from build123d import *

# Parameters (mm, degrees)
BOSS_EXTRUDE1_DEPTH = 8
CHAMFER1_SIZE       = 15


with BuildPart() as part:
    # Sketch1 → Boss-Extrude1 (new, symmetric)
    with BuildSketch(Plane.XY):
        Polygon((0, 0), (0, 30), (340, 30), (340, 10), align=None)
    extrude(amount=BOSS_EXTRUDE1_DEPTH, both=True)

    # Chamfer1
    chamfer1_edges = [part.edges().sort_by_distance(p)[0] for p in [
        (0, 30, 0),
    ]]
    chamfer(chamfer1_edges, length=CHAMFER1_SIZE)


solid = part.part
Geometry check sheet. Reference: the model listing, model coordinates, mm. Give positions to 0.01 mm unless a question says otherwise; leave off trailing zeros. Write each loop counter-clockwise with the first axis right and the second up, starting at its lowest first coordinate (ties: lowest second). Pieces come first, ordered by that corner, then holes.
1) Thickness scan on line 1 (Y direction, x = 274, z = -3.75); line 2 (Y direction, x = 272.5, z = 0.5); line 3 (X direction, y = 18.25, z = 5.5). Record the ranges inside material, lowest first.
Values follow:
line 1: y = 8.06 to 30
line 2: y = 8.01 to 30
line 3: x = 3.25 to 340
2) Cross-section at C-C (z = 1.25). Record the boundary of the cut face in (x, y).
Values follow:
outline: (0, 0) - (340, 10) - (340, 30) - (15, 30) - (0, 15) - close
3) Cross-section at A-A (x = 42.5). Record the boundary of the cut face in (y, z).
Values follow:
outline: (1.25, -8) - (30, -8) - (30, 8) - (1.25, 8) - close
4) Go/stop test with flat-tipped pins: pin 1 Ø1 at (y, z) = (19, -0.5) entering from -X; pin 2 Ø8 at (x, z) = (241, 1.5) entering from -Y. Record where each tip stops, or that it passes through.
Values follow:
pin 1: stops at x = 3.5
pin 2: stops at y = 6.97
5) Cross-section at B-B (y = 23). Record the boundary of the cut face in (x, z).
Values follow:
outline: (8, -8) - (340, -8) - (340, 8) - (8, 8) - close
